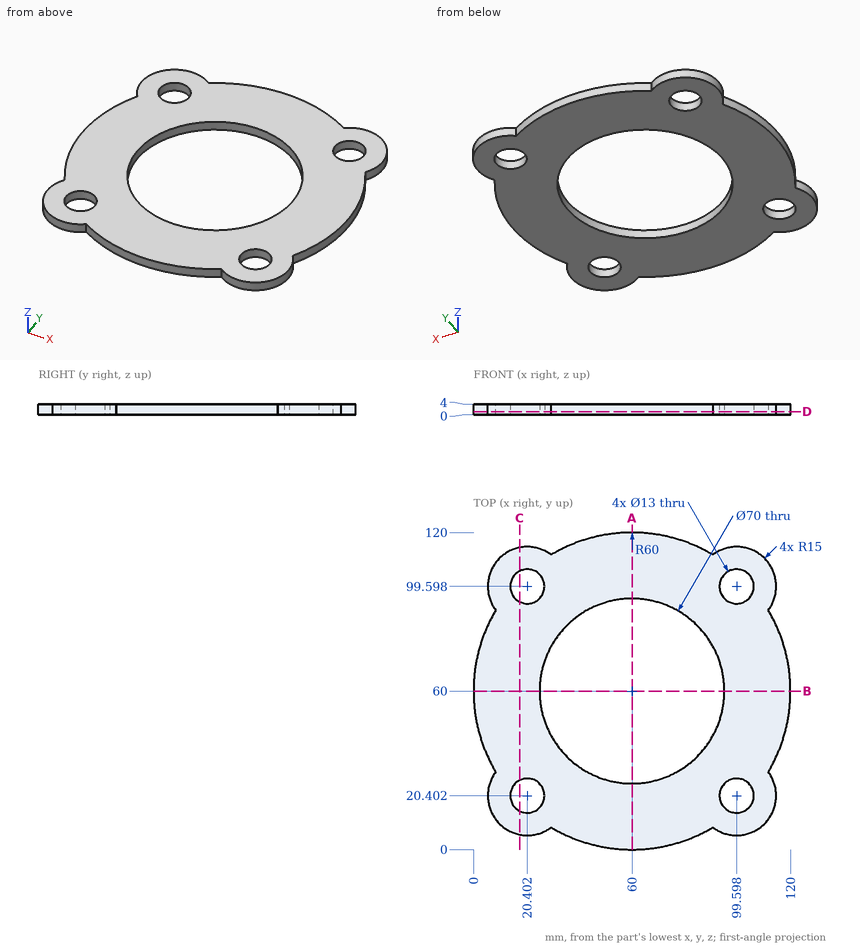
Input: dimensioned drawing with shaded views. Units: mm. Origin: part minimum x, y, z. Coordinates: 2 decimals unless noted, no trailing zeros. Order: outer loops, then holes, each group sorted by start corner. A loop starts at its lowest first (then second) coordinate and runs counter-clockwise, first axis right, second up. Notation, with made-up numbers: (-40, 30) -> (-18, 30) arc R31 ccw to (-18, 65) -> close; hole circle Ø5 at (31.5, -13). An arc over 180 degrees is marked (long way). Answer in a Markdown table with one row per item.
Item 1: Section C-C on x = 17.5. Output: boundary loops of the cut face in (y, z), plus the area to 3 significant figures.
Return value:
| item | result |
|---|---|
| outline | (5.69, 0) -> (14.59, 0) -> (14.59, 4) -> (5.69, 4) -> close; (26.22, 0) -> (93.78, 0) -> (93.78, 4) -> (26.22, 4) -> close; (105.41, 0) -> (114.31, 0) -> (114.31, 4) -> (105.41, 4) -> close |
| area | 341 mm² |
Item 2: Contact query for flat-ended pins moving along their axis: P1, Ø1, axis at y = 57.5, z = 0.5, coming from the -X side; P2, Ø1, axis at x = 47, z = 1, coming from the -Y side; P3, Ø1.5, axis at x = 83.5, z = 2, coming from the +Y side; P4, Ø10.5, axis at x = 20.4, y = 99.6, coming from the +Z side. Output: stop coordinate, or through.
Return value:
| item | result |
|---|---|
| P1 | stops at x = 0.03 |
| P2 | stops at y = 1.32 |
| P3 | stops at y = 115.52 |
| P4 | passes through |
Item 3: Section D-D on z = 1.15. Output: boundary loops of the cut face in (x, y), plus the area to 3 significant figures.
Return value:
| item | result |
|---|---|
| outline | (8.39, 29.39) arc R15 ccw to (29.39, 8.39) arc R60 ccw to (90.61, 8.39) arc R15 ccw to (111.61, 29.39) arc R60 ccw to (111.61, 90.61) arc R15 ccw to (90.61, 111.61) arc R60 ccw to (29.39, 111.61) arc R15 ccw to (8.39, 90.61) arc R60 ccw to start; hole circle Ø13 at (20.4, 20.4); hole circle Ø13 at (20.4, 99.6); hole circle Ø70 at (60, 60); hole circle Ø13 at (99.6, 20.4); hole circle Ø13 at (99.6, 99.6) |
| area | 7,940 mm² |
Item 4: Section A-A on x = 60. Output: boundary loops of the cut face in (y, z), plus the area to 3 significant figures.
Return value:
| item | result |
|---|---|
| outline | (0, 0) -> (25, 0) -> (25, 4) -> (0, 4) -> close; (95, 0) -> (120, 0) -> (120, 4) -> (95, 4) -> close |
| area | 200 mm² |
Item 5: Ray query, L1, parallel to Y at x = 60, z = 1; L2, parallel to Y at x = 20.5, z = 0.8; L3, parallel to X at y = 101, z = 1.55 (3 decimals). Return the intervals inside material, ascending.
Return value:
| item | result |
|---|---|
| L1 | y = 0 to 25, 95 to 120 |
| L2 | y = 5.4 to 13.9, 26.9 to 93.1, 106.1 to 114.6 |
| L3 | x = 5.468 to 14.055, 26.749 to 93.251, 105.945 to 114.532 |
